Input: dimensioned drawing with shaded views. Units: mm. Origin: part minimum x, y, z. Round coordinates to 2 decimals unless told otherwise and drop trailing zeros. Order: outer loops, then holes, each group sorted by start corner. A loop starts at its lowest first (then second) coordinate and runs counter-clockwise, first axis right, second up. Notation, with made-up numbers: M -4.75,16.25 L 18.25,16.25 A19 ccw 18.25,32.25 Z; hole C -29.5,89.5 d9. An arc over 180 degrees is marked long. Use CSV: the item, a comma, the result in double quotes. Start each with the question number.
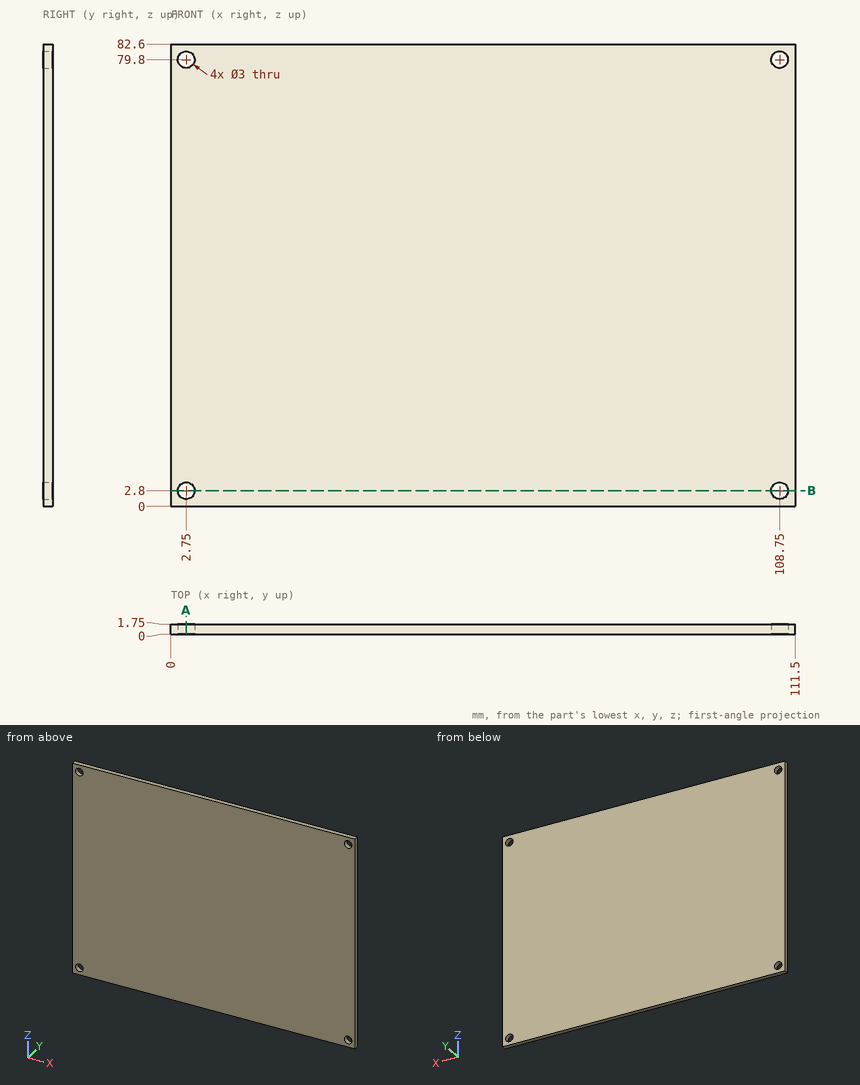
(1) Section A-A on x = 2.75. Return loops of the section in (y, z).
(2) Section B-B on z = 2.8. Return loops of the section in (x, y).
(3) Line query: line 1 along Z through (x, y) = (108.75, 1.2); line 2 along X through (y, z) = (0.55, 79.8). Output: solid intervals per line, ascending.
(4) Contact query for a flat-ended pin moving along its axis: P1, Ø1.8, axis at x = 108.75, z = 79.8, coming from the -Y side. Output: stop coordinate, or through.
Results below:
1,outline,"M 0,0 L 1.75,0 L 1.75,1.3 L 0,1.3 Z; M 0,4.3 L 1.75,4.3 L 1.75,78.3 L 0,78.3 Z; M 0,81.3 L 1.75,81.3 L 1.75,82.6 L 0,82.6 Z"
2,outline,"M 0,0 L 1.25,0 L 1.25,1.75 L 0,1.75 Z; M 4.25,0 L 107.25,0 L 107.25,1.75 L 4.25,1.75 Z; M 110.25,0 L 111.5,0 L 111.5,1.75 L 110.25,1.75 Z"
3,line 1,"z = 0 to 1.3, 4.3 to 78.3, 81.3 to 82.6"
3,line 2,"x = 0 to 1.25, 4.25 to 107.25, 110.25 to 111.5"
4,P1,"passes through"
